from build123d import *

# Parameters (mm, degrees)
SKETCH_1_W      = 45
SKETCH_1_H      = 58
SKETCH_1_R      = 8.5
EXTRUDE_1_DEPTH = 6
SKETCH_2_W      = 45
SKETCH_2_H      = 14
EXTRUDE_2_DEPTH = 12
M8X1_0_1_D      = 7
FILLET_1_R      = 2


with BuildPart() as part:
    # 草图1 → 凸台-拉伸1 (new body)
    with BuildSketch(Plane.XY):
        with Locations((0, -17)):
            Rectangle(SKETCH_1_W, SKETCH_1_H)
        Circle(SKETCH_1_R, mode=Mode.SUBTRACT)
    extrude_1 = extrude(amount=EXTRUDE_1_DEPTH)

    # 草图2 → 凸台-拉伸2 (add)
    with BuildSketch(Plane(origin=(0, 0, 0), x_dir=(-1, 0, 0), z_dir=(0, 0, -1))):
        with Locations((0, -39)):
            Rectangle(SKETCH_2_W, SKETCH_2_H)
    extrude(amount=EXTRUDE_2_DEPTH)

    # M8x1.0 螺纹孔1 (through all)
    with Locations(Plane(origin=(15.5, -12, 6), x_dir=(1, 0, 0), z_dir=(0, 0, 1))):
        with Locations((0, 0)):
            m8x1_0_1 = Hole(M8X1_0_1_D / 2)

    # 镜向1: 凸台-拉伸1, M8x1.0 螺纹孔1 across plane
    add(extrude_1.mirror(Plane(origin=(0, -39, 0), x_dir=(0, 0, 1), z_dir=(0, -1, 0))))
    add(m8x1_0_1.mirror(Plane(origin=(0, -39, 0), x_dir=(0, 0, 1), z_dir=(0, -1, 0))), mode=Mode.SUBTRACT)

    # 圆角1
    fillet_1_edges = [part.edges().sort_by_distance(p)[0] for p in [
        (22.5, -90, 3),
        (-22.5, -90, 3),
        (-22.5, 12, 3),
        (22.5, 12, 3),
    ]]
    fillet(fillet_1_edges, radius=FILLET_1_R)


solid = part.part
Input: part model. Units: mm. Frame: model coordinates. A direction names the side the tool comes from. Coordinates: 2 decimals unless noted, no trailing zeros. Order: outer loops, then holes, each group sorted by start corner. A loop starts at its lowest first (then second) coordinate and runs counter-clockwise, first axis right, second up. Notation, with made-up numbers: M 18,74.5 L 40,74.5 A31 cw 40,107.5 Z; hole C -6,25 d5. An arc over 180 degrees is marked long. Answer in a Markdown table with one row per item.
(1) Section query A-A, the plane x = 15.5. Output: boundary loops of the cut face in (y, z), plus the area to 3 significant figures.
Numbers:
| item | result |
|---|---|
| outline | M -90,0 L -69.5,0 L -69.5,6 L -90,6 Z; M -62.5,0 L -46,0 L -46,-12 L -32,-12 L -32,0 L -15.5,0 L -15.5,6 L -62.5,6 Z; M -8.5,0 L 12,0 L 12,6 L -8.5,6 Z |
| area | 696 mm^2 |
(2) Contact query for flat-ended pins moving along their axis: pin 1 Ø1.5 at (x, y) = (5.5, -6.5) entering from -Z; pin 2 Ø6 at (x, z) = (2.5, -5.5) entering from +Y; pin 3 Ø6 at (x, z) = (-5.5, -6.5) entering from -Y. Output: stop coordinate, or through.
Numbers:
| item | result |
|---|---|
| pin 1 | stops at z = 0 |
| pin 2 | stops at y = -32 |
| pin 3 | stops at y = -46 |
(3) Material intervals for line 1 (Y direction, x = 15.5, z = 3.65); line 2 (Y direction, x = 0, z = 1.7); line 3 (X direction, y = -78, z = 5), sorted ascending. Write a range as [from, to].
Numbers:
| item | result |
|---|---|
| line 1 | y = [-90, -69.5], [-62.5, -15.5], [-8.5, 12] |
| line 2 | y = [-90, -86.5], [-69.5, -8.5], [8.5, 12] |
| line 3 | x = [-22.5, -8.5], [8.5, 22.5] |
(4) Section query D-D, the plane x = 9.5. Output: boundary loops of the cut face in (y, z).
Numbers:
| item | result |
|---|---|
| outline | M -90,0 L -46,0 L -46,-12 L -32,-12 L -32,0 L 12,0 L 12,6 L -90,6 Z |
(5) Section query C-C, the plane z = 4. Output: boundary loops of the cut face in (x, y).
Numbers:
| item | result |
|---|---|
| outline | M -22.5,-88 A2 ccw -20.5,-90 L 20.5,-90 A2 ccw 22.5,-88 L 22.5,10 A2 ccw 20.5,12 L -20.5,12 A2 ccw -22.5,10 Z; hole C 0,-78 d17; hole C 0,0 d17; hole C 15.5,-66 d7; hole C 15.5,-12 d7 |
(6) Draft query along X for faces 1 (the cylindrical face through (13.885, -15.105, 2.958)), 2 (the flat face through (0, -39, -12)), 3 (the cylindrical face through (21.93, 11.4, 3.04)). Return one class per face: pulls with the +X half, pulls with the -X half, needs draft (parallel to the pull), parting line crosses it, or undercut.
Numbers:
| item | result |
|---|---|
| face 1 | undercut |
| face 2 | needs draft |
| face 3 | pulls with the +X half |
(7) Access query for faces 4 (the flat face through (0, -46, -6)), 5 (the flat face through (0, -32, -6)), 6 (the flat face through (22.5, -40, 1)). Directions: +Z, -Z, +X, -X, +Y, -Y. A direction counts if a zero-diameter tool reaches every point of the face in a straight line with its end or side. Return the directions, or none.
Numbers:
| item | result |
|---|---|
| face 4 | -Z, +X, -X, -Y |
| face 5 | -Z, +X, -X, +Y |
| face 6 | +Z, -Z, +X, +Y, -Y |
(8) Section query B-B, the plane y = -12. Output: boundary loops of the cut face in (x, z), plus the area to 3 significant figures.
Numbers:
| item | result |
|---|---|
| outline | M -22.5,0 L 12,0 L 12,6 L -22.5,6 Z; M 19,0 L 22.5,0 L 22.5,6 L 19,6 Z |
| area | 228 mm^2 |
